Source: CAD feature listing. Evaluate the final solid. Frame: model axes, mm. A direction names the side the tool comes from. Give positions to 0.01 mm unless a question says otherwise; leave off trailing zeros. Order: outer loops, then holes, each group sorted by start corner. A loop starts at its lowest first (then second) coordinate and runs counter-clockwise, first axis right, second up.
from build123d import *

# Parameters (mm, degrees)
BASE_PLATE_DEPTH   = 9
BASE_SLOT_DEPTH    = 28
CLEVIS_EAR_1_DEPTH = 9
CLEVIS_START       = -9
CLEVIS_EAR_2_DEPTH = 9
PIN_HOLE_SKETCH_R  = 7
PIN_HOLE_DEPTH     = 80


with BuildPart() as part:
    # Base Plate Sketch → Base Plate (new body)
    with BuildSketch(Plane(origin=(0, 0, 0), x_dir=(-1, 0, 0), z_dir=(0, 0, 1))):
        with BuildLine():
            Line((0, 0), (86, 0))
            ThreePointArc((86, 0), (106, 20), (86, 40))
            Line((86, 40), (0, 40))
            Line((0, 40), (0, 0))
        make_face()
    extrude(amount=BASE_PLATE_DEPTH)

    # Base Slot Sketch → Base Slot (cut)
    with BuildSketch(Plane(origin=(0, 0, 0), x_dir=(1, 0, 0), z_dir=(0, 0, -1))):
        with BuildLine():
            Line((-86, 27), (-63, 27))
            ThreePointArc((-63, 27), (-56, 20), (-63, 13))
            Line((-63, 13), (-86, 13))
            ThreePointArc((-86, 13), (-93, 20), (-86, 27))
        make_face()
    extrude(amount=-BASE_SLOT_DEPTH, mode=Mode.SUBTRACT)

    # Clevis Ear 1 Sketch → Clevis Ear 1 (add)
    with BuildSketch(Plane.XZ.offset(40)):
        with BuildLine():
            Line((0, 9), (0, 38))
            ThreePointArc((0, 38), (-17.5, 55.5), (-35, 38))
            Line((-35, 38), (-35, 9))
            Line((-35, 9), (0, 9))
        make_face()
    extrude(amount=-CLEVIS_EAR_1_DEPTH)

    # Clevis Ear 2 Sketch → Clevis Ear 2 (add)
    with BuildSketch(Plane(origin=(0, 0, 0), x_dir=(-1, 0, 0), z_dir=(0, 1, 0)).offset(CLEVIS_START)):
        with BuildLine():
            Line((0, 9), (0, 38))
            ThreePointArc((0, 38), (17.5, 55.5), (35, 38))
            Line((35, 38), (35, 9))
            Line((35, 9), (0, 9))
        make_face()
    extrude(amount=CLEVIS_EAR_2_DEPTH)

    # Pin Hole Sketch → Pin Hole (cut)
    with BuildSketch(Plane(origin=(0, 0, 0), x_dir=(-1, 0, 0), z_dir=(0, 1, 0))):
        with Locations(Location((17.5, 38, 0), (0, 0, 90))):
            Circle(PIN_HOLE_SKETCH_R)
    extrude(amount=-PIN_HOLE_DEPTH, mode=Mode.SUBTRACT)


solid = part.part
1) Section query B-B on x = -17.5. Output: boundary loops of the cut face in (y, z), and give its area (3 significant figures).
Checks:
outline: (-40, 0) - (0, 0) - (0, 31) - (-9, 31) - (-9, 9) - (-31, 9) - (-31, 31) - (-40, 31) - close; (-40, 45) - (-31, 45) - (-31, 55.5) - (-40, 55.5) - close; (-9, 45) - (0, 45) - (0, 55.5) - (-9, 55.5) - close
area: 945 mm2
2) Reachability of faces 1 (the face through (-18, -31, 27)), 2 (the face through (-35, -36, 24)), 3 (the face through (-74, -13, 4)) from +Z, -Z, +X, -X, +Y, -Y: full face, straight path, thin tool, end or side. Return the list, or none.
Checks:
face 1: +Z, +X, -X
face 2: +Z, -X, +Y, -Y
face 3: +Z, -Z
3) Section query C-C on y = -20. Output: boundary loops of the cut face in (x, z).
Checks:
outline: (-106, 0) - (-93, 0) - (-93, 9) - (-106, 9) - close; (-56, 0) - (0, 0) - (0, 9) - (-56, 9) - close
4) First-contact query: pin 1 Ø12 at (y, z) = (-9, 34.5) entering from -X; pin 2 Ø1.5 at (x, y) = (-47.5, -8) entering from +Z; pin 3 Ø1 at (y, z) = (-33, 40) entering from -X. Flat tips, straight axial feed; report the tip coordinate or a pass-through.
Checks:
pin 1: stops at x = -35
pin 2: stops at z = 9
pin 3: stops at x = -34.94
5) Ray query, L1, parallel to Z at x = -17, y = -5; L2, parallel to X at y = -34, z = 38; L3, parallel to Y at x = -22.5, z = 50. Return the intervals inside material, ascending.
Checks:
L1: z = 0 to 31.02, 44.98 to 55.49
L2: x = -35 to -24.5, -10.5 to 0
L3: y = -40 to -31, -9 to 0
6) Pull-direction query (Y, two-part tool) for faces 4 (the face through (-24, 0, 22)), 5 (the face through (-75, -27, 4)), 6 (the face through (0, -20, 6)); classes: +Y half, -Y half, draft (parallel to the pull), parting line (faces both ways), or undercut.
Checks:
face 4: +Y half
face 5: undercut
face 6: draft
7) Section query A-A on z = 19.5. Output: boundary loops of the cut face in (x, y).
Checks:
outline: (-35, -40) - (0, -40) - (0, -31) - (-35, -31) - close; (-35, -9) - (0, -9) - (0, 0) - (-35, 0) - close
8) Section query D-D on y = -33.5. Output: boundary loops of the cut face in (x, z), and give its area (3 significant figures).
Checks:
outline: (-100.76, 0) - (0, 0) - (0, 38) arc R17.5 ccw to (-35, 38) - (-35, 9) - (-100.76, 9) - close; hole circle Ø14 at (-17.5, 38)
area: 2,250 mm2
